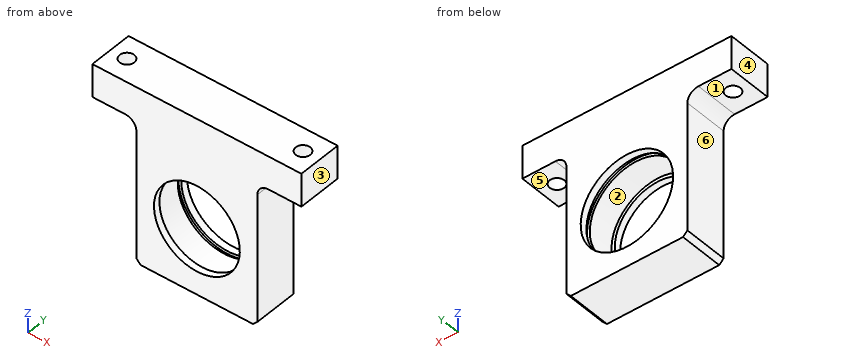
```python
from build123d import *

# Parameters (mm, degrees)
SKETCH_1_R          = 21
EXTRUDE_1_DEPTH     = 20
CHAMFER_1_SIZE      = 2
FILLET_1_R          = 5
SKETCH_2_R          = 21
SKETCH_2_R_2        = 19.5
EXTRUDE_2_DEPTH     = 3
HOLE_WIZARD_M6_1_D  = 6.6
SKETCH_9_R          = 22.25
SKETCH_9_R_2        = 21
CUT_EXTRUDE_1_DEPTH = 1.85


with BuildPart() as part:
    # 草图1 → 凸台-拉伸1 (new body)
    with BuildSketch(Plane(origin=(0, 0, 0), x_dir=(1, 0, 0), z_dir=(0, 1, 0))):
        Polygon((-47.5, 0), (47.5, 0), (47.5, 15), (27.5, 15), (27.5, 80), (-27.5, 80), (-27.5, 15), (-47.5, 15), align=None)
        with Locations(Location((0, 50, 0), (0, 0, 270))):
            Circle(SKETCH_1_R, mode=Mode.SUBTRACT)
    extrude(amount=EXTRUDE_1_DEPTH)

    # 倒角1
    chamfer_1_edges = [part.edges().sort_by_distance(p)[0] for p in [
        (-27.5, 10, -80),
        (27.5, 10, -80),
    ]]
    chamfer(chamfer_1_edges, length=CHAMFER_1_SIZE)

    # 圆角1
    fillet_1_edges = [part.edges().sort_by_distance(p)[0] for p in [
        (-27.5, 10, -15),
        (27.5, 10, -15),
    ]]
    fillet(fillet_1_edges, radius=FILLET_1_R)

    # 草图2 → 凸台-拉伸2 (add)
    with BuildSketch(Plane.XZ):
        with Locations(Location((0, -50, 0), (0, 0, 270))):
            Circle(SKETCH_2_R)
        with Locations(Location((0, -50, 0), (0, 0, 270))):
            Circle(SKETCH_2_R_2, mode=Mode.SUBTRACT)
    extrude(amount=-EXTRUDE_2_DEPTH)

    # M6 间隙孔1 (through all)
    with Locations(Plane(origin=(0, 0, -15), x_dir=(-1, 0, 0), z_dir=(0, 0, -1))):
        with Locations((-40, 10), (40, 10)):
            Hole(HOLE_WIZARD_M6_1_D / 2)

    # 草图9 → 切除-拉伸1 (cut)
    with BuildSketch(Plane(origin=(0, 15, 0), x_dir=(1, 0, 0), z_dir=(0, 1, 0))):
        with Locations(Location((0, 50, 0), (0, 0, 270))):
            Circle(SKETCH_9_R)
        with Locations(Location((0, 50, 0), (0, 0, 90))):
            Circle(SKETCH_9_R_2, mode=Mode.SUBTRACT)
    extrude(amount=CUT_EXTRUDE_1_DEPTH, mode=Mode.SUBTRACT)


solid = part.part
```
Geometry: final body of the model. Coordinates: model frame, mm. Face numbers are marked on the shaded views. A direction names the side the tool comes from. Round coordinates to 2 decimals unless told otherwise and drop trailing zeros. Write each loop counter-clockwise with the first axis right and the second up, starting at its lowest first coordinate (ties: lowest second). Pieces come first, ordered by that corner, then holes. Notation, with made-up numbers: M -37.75,54.5 L 14.25,54.5 A12 cw 14.25,67.5 Z; hole C -18,16 d9. An arc over 180 degrees is marked long. Answer in a Markdown table with one row per item. Add a question column.
(1) Cut plane A-A, the plane y = 10. Return the cut outline in (x, z).
(2) Cut plane D-D, the plane x = -40. Return the cut outline in (y, z).
(3) Contact query for flat-ended pins moving along their axis: pin 1 (6 mm diameter, centred on y = 5, z = -56.5, fed in from +X); pin 2 (1.5 mm diameter, centred on x = -17, z = -48.5, fed in from -Y); pin 3 (1.5 mm diameter, centred on x = -1, y = 7, fed in from +Z); pin 4 (10.5 mm diameter, centred on x = 40, y = 10, fed in from -Z). Output: stop coordinate, or through.
(4) Cut plane B-B, the plane x = 0. Return the cut outline in (y, z).
(5) Draft query along Z for the marked faces 1, 2 and 3. Return one class per face: pulls with the +Z half, pulls with the -Z half, needs draft (parallel to the pull), parting line crosses it, or undercut.
(6) Cut plane C-C, the plane z = -50. Return the cut outline in (x, y), then the cut area to 3 significant figures.
(7) Ray query, L1, parallel to Z at x = 0, y = 19; L2, parallel to X at y = 5.75, z = -50; L3, parallel to Y at x = -40, z = -6. Return the intervals inside material, ascending.
(8) Reachability of the marked faces 4, 5 and 6 from +Z, -Z, +X, -X, +Y, -Y: full face, straight path, thin tool, end or side. Return the list, or none.
Established:
| question | item | result |
|---|---|---|
| 1 | outline | M -47.5,-15 L -43.3,-15 L -43.3,0 L -47.5,0 Z; M -36.7,-15 L -32.5,-15 A5 cw -27.5,-20 L -27.5,-78 L -25.5,-80 L 25.5,-80 L 27.5,-78 L 27.5,-20 A5 cw 32.5,-15 L 36.7,-15 L 36.7,0 L -36.7,0 Z; M 43.3,-15 L 47.5,-15 L 47.5,0 L 43.3,0 Z; hole C 0,-50 d42 |
| 2 | outline | M 0,-15 L 6.7,-15 L 6.7,0 L 0,0 Z; M 13.3,-15 L 20,-15 L 20,0 L 13.3,0 Z |
| 3 | pin 1 | x = 27.5 |
| 3 | pin 2 | through |
| 3 | pin 3 | z = 0 |
| 3 | pin 4 | z = -15 |
| 4 | outline | M 0,-80 L 20,-80 L 20,-71 L 16.85,-71 L 16.85,-72.25 L 15,-72.25 L 15,-71 L 3,-71 L 3,-69.5 L 0,-69.5 Z; M 0,-30.5 L 3,-30.5 L 3,-29 L 15,-29 L 15,-27.75 L 16.85,-27.75 L 16.85,-29 L 20,-29 L 20,0 L 0,0 Z |
| 5 | face 1 | pulls with the -Z half |
| 5 | face 2 | undercut |
| 5 | face 3 | needs draft |
| 6 | outline | M -27.5,0 L -19.5,0 L -19.5,3 L -21,3 L -21,15 L -22.25,15 L -22.25,16.85 L -21,16.85 L -21,20 L -27.5,20 Z; M 19.5,0 L 27.5,0 L 27.5,20 L 21,20 L 21,16.85 L 22.25,16.85 L 22.25,15 L 21,15 L 21,3 L 19.5,3 Z |
| 6 | area | 264 mm² |
| 7 | L1 | -80 to -71, -29 to 0 |
| 7 | L2 | -27.5 to -21, 21 to 27.5 |
| 7 | L3 | 0 to 6.7, 13.3 to 20 |
| 8 | face 4 | +Z, -Z, -X, +Y, -Y |
| 8 | face 5 | -Z, +X, +Y, -Y |
| 8 | face 6 | -Z, -X, +Y, -Y |
